```python
from build123d import *

# Parameters (mm, degrees)
EXTRUDE_1_DEPTH = 10
SKETCH_2_W      = 10
SKETCH_2_H      = 125
EXTRUDE_2_DEPTH = 10
SKETCH_3_W      = 10
SKETCH_3_H      = 125
EXTRUDE_3_DEPTH = 10


with BuildPart() as part:
    # 草图1 → 凸台-拉伸1 (new body)
    with BuildSketch(Plane.XY):
        Polygon((0, 0), (460, 0), (460, -115), (410, -115), (410, -240), (50, -240), (50, -115), (0, -115), align=None)
    extrude(amount=EXTRUDE_1_DEPTH)

    # 草图2 → 凸台-拉伸2 (add)
    with BuildSketch(Plane(origin=(410, 0, 0), x_dir=(0, 0, -1), z_dir=(1, 0, 0))):
        with Locations((-5, -177.5)):
            Rectangle(SKETCH_2_W, SKETCH_2_H)
    extrude(amount=EXTRUDE_2_DEPTH)

    # 草图3 → 凸台-拉伸3 (add)
    with BuildSketch(Plane.ZY.offset(-50)):
        with Locations((5, -177.5)):
            Rectangle(SKETCH_3_W, SKETCH_3_H)
    extrude(amount=EXTRUDE_3_DEPTH)


solid = part.part
```
Source: CAD feature listing. Evaluate the final solid. Frame: model axes, mm. A direction names the side the tool comes from. Round coordinates to 2 decimals unless told otherwise and drop trailing zeros. Loops run counter-clockwise (first coordinate to the right, second up) from the corner with the lowest first, then second, coordinate; pieces in that order, holes last. Notation, with made-up numbers: M 67.25,-27 L 100.25,-27 A25 cw 100.25,-15 Z; hole C 7,23 d9. An arc over 180 degrees is marked long. Put each result on its own line as item: value.
(1) Section A-A, the plane z = 8.5. Return loops of the section in (x, y).
Solutions:
outline: M 0,-115 L 40,-115 L 40,-240 L 420,-240 L 420,-115 L 460,-115 L 460,0 L 0,0 Z
(2) Ray query, line 1 (X direction, y = -135.5, z = 8); line 2 (Y direction, x = 30, z = 1.75). Return the intervals inside material, ascending. Write a range as [from, to].
Solutions:
line 1: [40, 420]
line 2: [-115, 0]
(3) Access query for faces 1 (the face through (440, -115, 5)), 2 (the face through (40, -177, 5)), 3 (the face through (0, -58, 5)). Directions: +Z, -Z, +X, -X, +Y, -Y. A direction counts if a zero-diameter tool reaches every point of the face in a straight line with its end or side. Return the directions, or none.
Solutions:
face 1: +Z, -Z, +X, -Y
face 2: +Z, -Z, -X, -Y
face 3: +Z, -Z, -X, +Y, -Y
(4) First-contact query: pin 1 (4 mm diameter, centred on y = -185, z = 7.5, fed in from -X); pin 2 (3 mm diameter, centred on x = 23.5, z = 5.5, fed in from -Y). Flat tips, straight axial feed; report the tip coordinate or a pass-through.
Solutions:
pin 1: x = 40
pin 2: y = -115
(5) Section B-B, the plane y = -193.5. Return loops of the section in (x, z), and give its area (3 significant figures).
Solutions:
outline: M 40,0 L 420,0 L 420,10 L 40,10 Z
area: 3,800 mm²
